For this review, take the finished solid that the model builds, in its own axes (mm). Face numbers are marked on the shaded views. A direction names the side the tool comes from. Coordinates: 2 decimals unless noted, no trailing zeros. Order: outer loops, then holes, each group sorted by start corner. A loop starts at its lowest first (then second) coordinate and runs counter-clockwise, first axis right, second up. Notation, with made-up numbers: (54.25, -24.5) -> (89.25, -24.5) arc R18 cw to (89.25, -13.5) -> close; hole circle Ø1 at (37.5, 25). An arc over 180 degrees is marked (long way). Return JSON: item names as keys, results as strings. Group by question number.
Item 1: For line 1 along Y through (x, z) = (-6.5, 19); line 2 along Y through (x, z) = (0, 27.5); line 3 along Z through (x, y) = (-6, 95), list the stretches that pass through material, from the lowest coordinate up.
Item 2: Take a section at A-A (z = 23.5). Write out the cut boundary in (x, y).
Item 3: Insertion check: pin 1 (3 mm diameter, centred on x = 17.5, z = 22.5, fed in from +Y); pin 2 (9 mm diameter, centred on x = -10, y = 112.36, fed in from -Z); pin 3 (9.5 mm diameter, centred on x = 2, z = 23.5, fed in from -Y); pin 4 (1 mm diameter, centred on x = 11.5, z = 26.5, fed in from -Y). Each pin has a flat end and moves straight along its axis. Give the tip position at first contact, or say it passes through.
Item 4: Take a section at D-D (x = 22). Write out the cut boundary in (y, z), then the cut area to 3 significant figures.
Item 5: Take a section at C-C (x = 0). Write out the cut boundary in (y, z).
Item 6: Machinability: for the marked faces 1, 2 and 3, which of the approach directions +Z, -Z, +X, -X, +Y, -Y give a long, thin tool a straight path to every point of the face, cutting with its end or side? Answer none if there is none.
Item 7: Take a section at B-B (y = 0). Write out the cut boundary in (x, z), then the cut area to 3 significant figures.
Item 8: Draft analysis for pull direction Y (two halves, no side actions). For the marked faces 4, 5 and 6, state which applies: +Y half, -Y half, draft (parallel to the pull), parting line (faces both ways), or undercut.
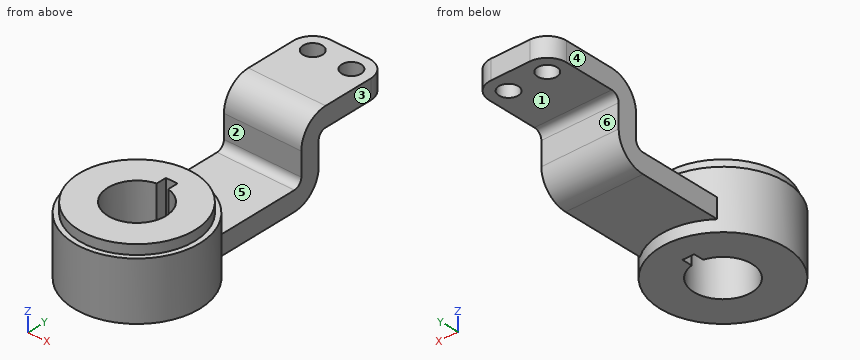
```python
from build123d import *

# Parameters (mm, degrees)
KEYED_HUB_PROFILE_R             = 32.5
KEYED_HUB_65_DEPTH              = 30
HUB_SHOULDER_PROFILE_R          = 30
HUB_SHOULDER_RING_60_DEPTH      = 5
SUPPORT_ARM_PROFILE_W           = 40
SUPPORT_ARM_PROFILE_H           = 60
SUPPORT_ARM_DEPTH               = 10
ARM_JOGGLE_PROFILE_W            = 40
ARM_JOGGLE_PROFILE_H            = 40
ARM_JOGGLE_DEPTH                = 10
MOUNTING_FLANGE_PROFILE_W       = 10
MOUNTING_FLANGE_PROFILE_H       = 50
MOUNTING_FLANGE_DEPTH           = 40
FLANGE_CORNER_FILLETS_R10_R     = 10
ARM_OUTER_BEND_FILLET_R14_R     = 14
JOGGLE_OUTER_BEND_FILLET_R14_R  = 14
ARM_JOGGLE_INNER_FILLET_R4_R    = 4
ARM_FLANGE_INNER_FILLET_R4_R    = 4
FLANGE_MOUNTING_HOLES_PROFILE_R = 5
FLANGE_MOUNTING_HOLES_2X_DEPTH  = 40


with BuildPart() as part:
    # Keyed Hub Profile → Keyed Hub Ø65 (new body)
    with BuildSketch(Plane.XY):
        Circle(KEYED_HUB_PROFILE_R)
        with BuildLine():
            Line((-3, 20), (3, 20))
            Line((3, 20), (3, 14.696938457))
            ThreePointArc((3, 14.696938457), (0, -15), (-3, 14.696938457))
            Line((-3, 14.696938457), (-3, 20))
        make_face(mode=Mode.SUBTRACT)
    extrude(amount=KEYED_HUB_65_DEPTH)

    # Hub Shoulder Profile → Hub Shoulder Ring Ø60 (add)
    with BuildSketch(Plane.XY.offset(30)):
        Circle(HUB_SHOULDER_PROFILE_R)
        with BuildLine():
            Line((-3, 14.696938457), (-3, 20))
            Line((-3, 20), (3, 20))
            Line((3, 20), (3, 14.696938457))
            ThreePointArc((3, 14.696938457), (0, -15), (-3, 14.696938457))
        make_face(mode=Mode.SUBTRACT)
    extrude(amount=HUB_SHOULDER_RING_60_DEPTH)

    # Support Arm Profile → Support Arm (add)
    with BuildSketch(Plane.XY.offset(6)):
        with Locations((0, 52.360679775)):
            Rectangle(SUPPORT_ARM_PROFILE_W, SUPPORT_ARM_PROFILE_H)
    extrude(amount=SUPPORT_ARM_DEPTH)

    # Arm Joggle Profile → Arm Joggle (add)
    with BuildSketch(Plane(origin=(0, 82.360679775, 0), x_dir=(1, 0, 0), z_dir=(0, 1, 0))):
        with Locations((0, -26)):
            Rectangle(ARM_JOGGLE_PROFILE_W, ARM_JOGGLE_PROFILE_H)
    extrude(amount=-ARM_JOGGLE_DEPTH)

    # Mounting Flange Profile → Mounting Flange (add)
    with BuildSketch(Plane(origin=(20, 0, 0), x_dir=(0, 0, -1), z_dir=(1, 0, 0))):
        with Locations((-41, 97.360679775)):
            Rectangle(MOUNTING_FLANGE_PROFILE_W, MOUNTING_FLANGE_PROFILE_H)
    extrude(amount=-MOUNTING_FLANGE_DEPTH)

    # Flange Corner Fillets R10
    flange_corner_fillets_r10_edges = [part.edges().sort_by_distance(p)[0] for p in [
        (20, 122.360679775, 41),
        (-20, 122.360679775, 41),
    ]]
    fillet(flange_corner_fillets_r10_edges, radius=FLANGE_CORNER_FILLETS_R10_R)

    # Arm Outer Bend Fillet R14
    arm_outer_bend_fillet_r14_edges = [part.edges().sort_by_distance(p)[0] for p in [
        (0, 82.360679775, 6),
    ]]
    fillet(arm_outer_bend_fillet_r14_edges, radius=ARM_OUTER_BEND_FILLET_R14_R)

    # Joggle Outer Bend Fillet R14
    joggle_outer_bend_fillet_r14_edges = [part.edges().sort_by_distance(p)[0] for p in [
        (0, 72.360679775, 46),
    ]]
    fillet(joggle_outer_bend_fillet_r14_edges, radius=JOGGLE_OUTER_BEND_FILLET_R14_R)

    # Arm-Joggle Inner Fillet R4
    arm_joggle_inner_fillet_r4_edges = [part.edges().sort_by_distance(p)[0] for p in [
        (0, 72.360679775, 16),
    ]]
    fillet(arm_joggle_inner_fillet_r4_edges, radius=ARM_JOGGLE_INNER_FILLET_R4_R)

    # Arm-Flange Inner Fillet R4
    arm_flange_inner_fillet_r4_edges = [part.edges().sort_by_distance(p)[0] for p in [
        (0, 82.360679775, 36),
    ]]
    fillet(arm_flange_inner_fillet_r4_edges, radius=ARM_FLANGE_INNER_FILLET_R4_R)

    # Flange Mounting Holes Profile → Flange Mounting Holes 2x (cut)
    with BuildSketch(Plane.XY.offset(46)):
        with Locations((-10, 112.360679775)):
            Circle(FLANGE_MOUNTING_HOLES_PROFILE_R)
        with Locations((10, 112.360679775)):
            Circle(FLANGE_MOUNTING_HOLES_PROFILE_R)
    extrude(amount=-FLANGE_MOUNTING_HOLES_2X_DEPTH, mode=Mode.SUBTRACT)


solid = part.part
```
Findings below:
{
 "1": {"line 1": "y = -31.84 to -13.52, 13.52 to 31.84, 72.23 to 82.32", "line 2": "y = -32.5 to -15, 20 to 32.5, 72.36 to 82.36", "line 3": "z = 36 to 46"},
 "2": {"outline": "circle Ø65 at (0, 0); (-20, 72.36) -> (20, 72.36) -> (20, 82.36) -> (-20, 82.36) -> close; hole (-3, 14.7) arc R15 ccw (long way) to (3, 14.7) -> (3, 20) -> (-3, 20) -> close"},
 "3": {"pin 1": "stops at y = 82.36", "pin 2": "passes through", "pin 3": "stops at y = -32.5", "pin 4": "stops at y = -30.58"},
 "4": {"outline": "(-23.92, 0) -> (23.92, 0) -> (23.92, 30) -> (20.4, 30) -> (20.4, 35) -> (-20.4, 35) -> (-20.4, 30) -> (-23.92, 30) -> close", "area": "1,640 mm2"},
 "5": {"outline": "(-32.5, 0) -> (-15, 0) -> (-15, 35) -> (-30, 35) -> (-30, 30) -> (-32.5, 30) -> close; (20, 0) -> (32.5, 0) -> (32.5, 6) -> (68.36, 6) arc R14 ccw to (82.36, 20) -> (82.36, 32) arc R4 cw to (86.36, 36) -> (122.36, 36) -> (122.36, 46) -> (86.36, 46) arc R14 ccw to (72.36, 32) -> (72.36, 20) arc R4 cw to (68.36, 16) -> (32.5, 16) -> (32.5, 30) -> (30, 30) -> (30, 35) -> (20, 35) -> close"},
 "6": {"face 1": "-Z, +X, -X, +Y", "face 2": "+Z, +X, -X", "face 3": "+Z, -Z, +X, +Y"},
 "7": {"outline": "(-32.5, 0) -> (-15, 0) -> (-15, 35) -> (-30, 35) -> (-30, 30) -> (-32.5, 30) -> close; (15, 0) -> (32.5, 0) -> (32.5, 30) -> (30, 30) -> (30, 35) -> (15, 35) -> close", "area": "1,200 mm2"},
 "8": {"face 4": "draft", "face 5": "undercut", "face 6": "+Y half"}
}
